Part model, mm, in its own coordinate system. A direction names the side the tool comes from. Give positions to 0.01 mm unless a question says otherwise; leave off trailing zeros. Order: outer loops, then holes, each group sorted by start corner. A loop starts at its lowest first (then second) coordinate and runs counter-clockwise, first axis right, second up. Notation, with made-up numbers: (46.25, 4) - (95.25, 4) arc R19 ccw to (95.25, 19) - close; hole circle Ø9 at (19.25, 62.5). An arc over 180 degrees is marked (long way). Use one line per item in the form item = value. Start each with the question number.
1. Band-saw the part on A-A, the plane x = 82. List the corners of the cut face in (y, z), plus the area to 3 significant figures.
2. Tool access for faces 1 (the face through (395.504, 11.923, -3.755)), 2 (the face through (-577.09, -2.17, 9.76)), 3 (the face through (3.14, -29.97, -1.32)): list every direction of +Z, -Z, +X, -X, +Y, -Y with a clear straight run to the whole face (end or side of a thin tool).
3. Band-saw the part on B-B, the plane x = -477. List the corners of the cut face in (y, z).
4. Drill centre lines: line 1 (Y direction, x = 635, z = 0); line 2 (Z direction, x = -80.5, y = -3). Where is each one in solid material? Low to high.
5. Pin check, flat tips, straight feed: P1, Ø1.5, axis at x = -63, z = -15.5, coming from the +Y side; P2, Ø3, axis at x = 275, z = -4, coming from the -Y side; P3, Ø10, axis at y = 23, z = 18, coming from the -X side; P4, Ø11, axis at y = 0, z = 0, coming from the +X side. Stop position of each tip, or through.
from build123d import *

# Parameters (mm, degrees)
CHAMFER_1_SIZE          = 1
HOLE_WIZARD_M10_1_D     = 8.5
HOLE_WIZARD_M10_1_DEPTH = 24.5
HOLE_WIZARD_M10_1_TIP   = 2.553657631


with BuildPart() as part:
    # 草图1 → 旋转1 (revolve)
    with BuildSketch(Plane.XY):
        Polygon((-593.3, 0), (-593.3, 10), (-562.3, 10), (-562.3, 12.5), (-225, 12.5), (-225, 30), (225, 30), (225, 12.5), (562.3, 12.5), (562.3, 10), (642.3, 10), (642.3, 0), align=None)
    revolve(axis=Axis((642.3, 0, 0), (-1, 0, 0)))

    # 倒角1
    chamfer_1_edges = [part.edges().sort_by_distance(p)[0] for p in [
        (225, -30, 0),
        (-225, -30, 0),
        (-562.3, -12.5, 0),
        (-593.3, -10, 0),
        (642.3, -10, 0),
        (562.3, -12.5, 0),
    ]]
    chamfer(chamfer_1_edges, length=CHAMFER_1_SIZE)

    # M10 螺纹孔1
    with Locations(Plane(origin=(642.3, 0, 0), x_dir=(0, 0, -1), z_dir=(1, 0, 0))):
        with Locations((0, 0)):
            Hole(HOLE_WIZARD_M10_1_D / 2, depth=HOLE_WIZARD_M10_1_DEPTH)
            with Locations((0, 0, -(HOLE_WIZARD_M10_1_DEPTH + HOLE_WIZARD_M10_1_TIP / 2))):  # 118° drill point
                Cone(0, HOLE_WIZARD_M10_1_D / 2, HOLE_WIZARD_M10_1_TIP, mode=Mode.SUBTRACT)


solid = part.part
From the geometry:
q1.outline = circle Ø60 at (0, 0)
q1.area = 2,830 mm²
q2.face_1 = +X
q2.face_2 = -X
q2.face_3 = +X, -X
q3.outline = circle Ø25 at (0, 0)
q4.line_1 = -10 to -4.25, 4.25 to 10
q4.line_2 = -29.85 to 29.85
q5.P1 = 26.12
q5.P2 = -12.25
q5.P3 = -225
q5.P4 = 642.3
